from build123d import *

# Parameters (mm, degrees)
SKETCH1_R           = 15
BOSS_EXTRUDE1_DEPTH = 6


with BuildPart() as part:
    # Sketch1 → Boss-Extrude1 (new, symmetric)
    with BuildSketch(Plane.XY):
        with BuildLine():
            Line((-26, 0), (-30, 0))
            Line((-30, 0), (-50, 20))
            Line((-50, 20), (-50, 57.5))
            ThreePointArc((-50, 57.5), (-49.701425001, 59.92535625), (-48.823529412, 62.205882353))
            Line((-48.823529412, 62.205882353), (-26.470588235, 104.117647059))
            ThreePointArc((-26.470588235, 104.117647059), (0, 120), (26.470588235, 104.117647059))
            Line((26.470588235, 104.117647059), (48.823529412, 62.205882353))
            ThreePointArc((48.823529412, 62.205882353), (49.701425001, 59.92535625), (50, 57.5))
            Line((50, 57.5), (50, 20))
            Line((50, 20), (30, 0))
            Line((30, 0), (26, 0))
            Line((26, 0), (26, 45))
            ThreePointArc((26, 45), (24.535533906, 48.535533906), (21, 50))
            Line((21, 50), (-21, 50))
            ThreePointArc((-21, 50), (-24.535533906, 48.535533906), (-26, 45))
            Line((-26, 45), (-26, 0))
        make_face()
        with Locations((0, 90)):
            Circle(SKETCH1_R, mode=Mode.SUBTRACT)
    extrude(amount=BOSS_EXTRUDE1_DEPTH, both=True)


solid = part.part
Model file for the job. Use its own axes, mm. A direction names the side the tool comes from. Give positions to 0.01 mm unless a question says otherwise; leave off trailing zeros. Order: outer loops, then holes, each group sorted by start corner. A loop starts at its lowest first (then second) coordinate and runs counter-clockwise, first axis right, second up. Notation, with made-up numbers: M 78,81.5 L 113,81.5 A13 cw 113,90.5 Z; hole C 43.5,18 d9. An arc over 180 degrees is marked long. Put each result on its own line as item: value. Start each with the question number.
(1) Pin check, flat tips, straight feed: pin 1 Ø3.5 at (y, z) = (12.5, 0.5) entering from +X; pin 2 Ø2 at (x, z) = (-33, -1) entering from +Y; pin 3 Ø2 at (x, z) = (37, -4) entering from +Y; pin 4 Ø1.5 at (x, y) = (21.5, 49.5) entering from +Z. Stop position of each tip, or through.
(2) Band-saw the part on A-A on x = 0. Give the cut face in (y, z), then the cut area to 3 significant figures.
(3) Tool access for faces 4 (the face through (-37.804, 82.868, 0.084)), 5 (the face through (-24, 49, 0)): list every direction of +Z, -Z, +X, -X, +Y, -Y with a clear straight run to the whole face (end or side of a thin tool).
(4) Band-saw the part on D-D on x = 28.5. Give the cut face in (y, z), then the cut area to 3 significant figures.
(5) Drill centre lines: L1, parallel to X at y = 35.5, z = 3.75; L2, parallel to Y at x = 0, z = 2.5; L3, parallel to X at y = 14, z = 1.5. Where is each one in solid material? Low to high. Write a range as [from, to].
(6) Pull direction X, two halves, no side cores. Call faces 1 (the face through (-26, 23, 0)), 2 (the face through (0, 120, 0)), 3 (the face through (-28, 0, 0)): released by +X, released by -X, zero draft, split by the parting line, or undercut.
(7) Band-saw the part on B-B on y = 90. Give the cut face in (x, z).
(8) Band-saw the part on C-C on z = -2.75. Give the cut face in (x, y), then the cut area to 3 significant figures.
Results below:
1. pin 1: stops at x = 44.25
1. pin 2: stops at y = 93.75
1. pin 3: stops at y = 86.25
1. pin 4: stops at z = 6
2. outline: M 50,-6 L 75,-6 L 75,6 L 50,6 Z; M 105,-6 L 120,-6 L 120,6 L 105,6 Z
2. area: 480 mm2
3. face 4: +Z, -Z, -X, +Y
3. face 5: +Z, -Z, -Y
4. outline: M 0,-6 L 100.31,-6 L 100.31,6 L 0,6 Z
4. area: 1,200 mm2
5. L1: x = [-50, -26], [26, 50]
5. L2: y = [50, 75], [105, 120]
5. L3: x = [-44, -26], [26, 44]
6. face 1: undercut
6. face 2: split by the parting line
6. face 3: zero draft
7. outline: M -34,-6 L -15,-6 L -15,6 L -34,6 Z; M 15,-6 L 34,-6 L 34,6 L 15,6 Z
8. outline: M -50,20 L -30,0 L -26,0 L -26,45 A5 cw -21,50 L 21,50 A5 cw 26,45 L 26,0 L 30,0 L 50,20 L 50,57.5 A10 ccw 48.82,62.21 L 26.47,104.12 A30 ccw -26.47,104.12 L -48.82,62.21 A10 ccw -50,57.5 Z; hole C 0,90 d30
8. area: 6,280 mm2
